```python
from build123d import *

# Parameters (mm, degrees)
SKETCH1_W             = 35
SKETCH1_H             = 32
BOSS_EXTRUDE1_DEPTH   = 20
CUT_EXTRUDE2_REACH    = 43.596
SKETCH3_R             = 3.25
SKETCH3_R_2           = 1.5
SKETCH4_R             = 1
CUT_EXTRUDE3_DEPTH    = 2
M3_TAPPED_HOLE1_D     = 2.5
M3_TAPPED_HOLE1_DEPTH = 7.5
M3_TAPPED_HOLE1_TIP   = 0.751075774


with BuildPart() as part:
    # Sketch1 → Boss-Extrude1 (new body)
    with BuildSketch(Plane(origin=(0, 0, 0), x_dir=(1, 0, 0), z_dir=(0, 1, 0))):
        Rectangle(SKETCH1_W, SKETCH1_H)
    extrude(amount=BOSS_EXTRUDE1_DEPTH)

    # Sketch3 → Cut-Extrude2 (cut, up to next)
    with BuildSketch(Plane.XY.offset(16), mode=Mode.PRIVATE) as cut_extrude2_sk1:
        with Locations((-2, 13.5)):
            Circle(SKETCH3_R)
    cut_extrude2_tool1 = extrude(cut_extrude2_sk1.sketch, amount=-CUT_EXTRUDE2_REACH, mode=Mode.PRIVATE) & part.part
    # Sketch3 → Cut-Extrude2 (cut, up to next)
    with BuildSketch(Plane.XY.offset(16), mode=Mode.PRIVATE) as cut_extrude2_sk2:
        with Locations((-2, 3.5)):
            Circle(SKETCH3_R_2)
    cut_extrude2_tool2 = extrude(cut_extrude2_sk2.sketch, amount=-CUT_EXTRUDE2_REACH, mode=Mode.PRIVATE) & part.part
    add(cut_extrude2_tool1.solids().sort_by_distance((-2, 13.5, 16))[0], mode=Mode.SUBTRACT)
    add(cut_extrude2_tool2.solids().sort_by_distance((-2, 3.5, 16))[0], mode=Mode.SUBTRACT)

    # Sketch4 → Cut-Extrude3 (cut)
    with BuildSketch(Plane(origin=(0, 20, 0), x_dir=(1, 0, 0), z_dir=(0, 1, 0))):
        with Locations(Location((-8, 1, 0), (0, 0, 270))):
            Circle(SKETCH4_R)
        with Locations(Location((-14.5, 1, 0), (0, 0, 270))):
            Circle(SKETCH4_R)
    extrude(amount=-CUT_EXTRUDE3_DEPTH, mode=Mode.SUBTRACT)

    # M3 Tapped Hole1
    with Locations(Plane(origin=(0, 20, 0), x_dir=(1, 0, 0), z_dir=(0, 1, 0))):
        with Locations((-8, 1), (-14.5, 1)):
            Hole(M3_TAPPED_HOLE1_D / 2, depth=M3_TAPPED_HOLE1_DEPTH)
            with Locations((0, 0, -(M3_TAPPED_HOLE1_DEPTH + M3_TAPPED_HOLE1_TIP / 2))):  # 118° drill point
                Cone(0, M3_TAPPED_HOLE1_D / 2, M3_TAPPED_HOLE1_TIP, mode=Mode.SUBTRACT)


solid = part.part
```
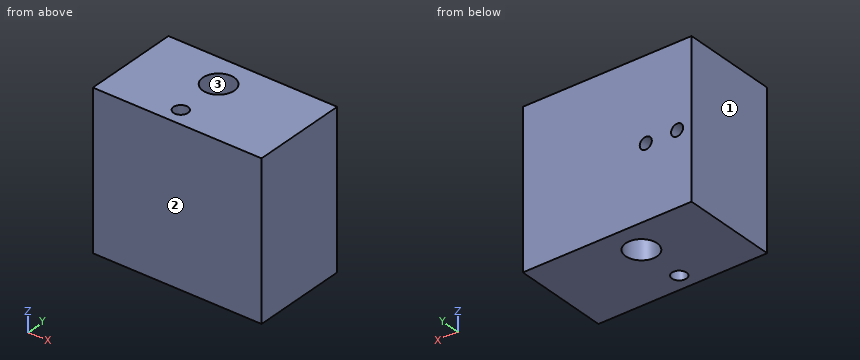
Read the model definition and answer for the solid it produces. Units are mm, in the model's axes. Face numbers are marked on the shaded views. Round coordinates to 2 decimals unless told otherwise and drop trailing zeros. Write each loop counter-clockwise with the first axis right and the second up, starting at its lowest first coordinate (ties: lowest second). Pieces come first, ordered by that corner, then holes. Notation, with made-up numbers: (34, 4) - (78, 4) arc R25 ccw to (78, 28) - close; hole circle Ø10 at (-30, -30.5). An arc over 180 degrees is marked (long way). One line per item, written item: value.
Q1. Straight lines are drawn through the part: line 1 (Y direction, x = -2, z = -8.5); line 2 (Z direction, x = -8, y = 17.75); line 3 (X direction, y = 2.5, z = -12). For each, find the intervals that lie inside material, in ascending order. Write a range as from..to.
The answers:
line 1: y = 0..2, 5..10.25, 16.75..20
line 2: z = -16..-2.25, 0.25..16
line 3: x = -17.5..-3.12, -0.88..17.5
Q2. Find section D-D (z = 4). Determine the outline of the cut face in (x, y).
The answers:
outline: (-17.5, 0) - (17.5, 0) - (17.5, 20) - (-17.5, 20) - close; hole circle Ø6.5 at (-2, 13.5); hole circle Ø3 at (-2, 3.5)
Q3. Find section B-B (x = -2). Determine the outline of the cut face in (y, z), and give its area (3 significant figures).
The answers:
outline: (0, -16) - (2, -16) - (2, 16) - (0, 16) - close; (5, -16) - (10.25, -16) - (10.25, 16) - (5, 16) - close; (16.75, -16) - (20, -16) - (20, 16) - (16.75, 16) - close
area: 336 mm2
Q4. Find section C-C (y = 3.5). Determine the outline of the cut face in (x, z).
The answers:
outline: (-17.5, -16) - (-3.5, -16) - (-3.5, 16) - (-17.5, 16) - close; (-0.5, -16) - (17.5, -16) - (17.5, 16) - (-0.5, 16) - close
Q5. Find section A-A (y = 13.5). Determine the outline of the cut face in (x, z).
The answers:
outline: (-17.5, -16) - (-5.25, -16) - (-5.25, 16) - (-17.5, 16) - close; (1.25, -16) - (17.5, -16) - (17.5, 16) - (1.25, 16) - close; hole circle Ø2.5 at (-14.5, -1); hole circle Ø2.5 at (-8, -1)
Q6. For a pull along X with two mould halves and no side action, classify the marked faces 1, 2 and 3 as pulls with the +X half, pulls with the -X half, needs draft (parallel to the pull), parting line crosses it, or undercut.
The answers:
face 1: pulls with the -X half
face 2: needs draft
face 3: undercut
